Read the model definition and answer for the solid it produces. Units are mm, in the model's axes. Coordinates: 2 decimals unless noted, no trailing zeros. Write each loop counter-clockwise with the first axis right and the second up, starting at its lowest first coordinate (ties: lowest second). Pieces come first, ordered by that corner, then holes. Notation, with made-up numbers: (6, 14.5) -> (23, 14.5) arc R18 cw to (23, 41.5) -> close; hole circle Ø7 at (31.25, 54.25). An arc over 180 degrees is marked (long way). Answer in a Markdown table with one row per item. Add a question column.
Item 1: Section A-A on x = -75 is taken. Write down the section's boundary in (y, z), then the cut area to 3 significant figures.
Item 2: Given pin 1 Ø8 at (x, y) = (89.5, 55) entering from +Z; pin 2 Ø3 at (x, y) = (-90.5, 54) entering from +Z, each flat-ended and moving along its own axis, determine where each tip first touches the part or whether it passes through.
Item 3: Straight lines are drawn through the part: line 1 (Y direction, x = -90, z = 8.3); line 2 (Y direction, x = 25, z = 5.75); line 3 (X direction, y = 40.35, z = 3.5). For each, find the intervals that lie inside material, in ascending order. Write a range as from..to.
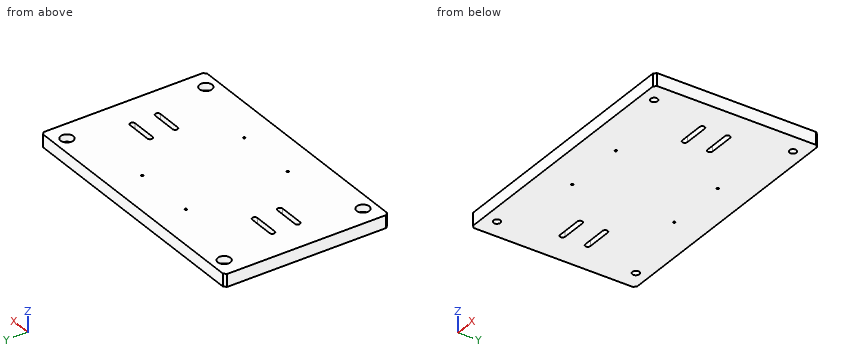
```python
from build123d import *

# Parameters (mm, degrees)
SKETCH1_W                                           = 210
SKETCH1_H                                           = 130
BOSS_EXTRUDE1_DEPTH                                 = 10
CUT_EXTRUDE1_DEPTH                                  = 124.895116934
CUT_EXTRUDE1_DEPTH_BACK                             = 124.895116934
HOLE_SIZE_PER_SOCKET_HEAD_CAP_SCREW_TYP_D           = 5.5
HOLE_SIZE_PER_SOCKET_HEAD_CAP_SCREW_TYP_CBORE_D     = 10
HOLE_SIZE_PER_SOCKET_HEAD_CAP_SCREW_TYP_CBORE_DEPTH = 5.7
M2_TAPPED_HOLE1_D                                   = 1.6
CHAMFER1_SIZE                                       = 2


with BuildPart() as part:
    # Sketch1 → Boss-Extrude1 (new body)
    with BuildSketch(Plane.XY):
        Rectangle(SKETCH1_W, SKETCH1_H)
    extrude(amount=BOSS_EXTRUDE1_DEPTH)

    # Sketch2 → Cut-Extrude1 (cut, two sides: drawn at the far end of the back side and taken through both)
    with BuildSketch(Plane.XY.offset(10).offset(-CUT_EXTRUDE1_DEPTH_BACK)):
        with BuildLine():
            Line((-80, 8), (-60, 8))
            ThreePointArc((-60, 8), (-58, 10), (-60, 12))
            Line((-60, 12), (-80, 12))
            ThreePointArc((-80, 12), (-82, 10), (-80, 8))
        make_face()
        with BuildLine():
            ThreePointArc((-60, -8), (-58, -10), (-60, -12))
            Line((-60, -12), (-80, -12))
            ThreePointArc((-80, -12), (-82, -10), (-80, -8))
            Line((-80, -8), (-60, -8))
        make_face()
        with BuildLine():
            Line((80, -8), (60, -8))
            ThreePointArc((60, -8), (58, -10), (60, -12))
            Line((60, -12), (80, -12))
            ThreePointArc((80, -12), (82, -10), (80, -8))
        make_face()
        with BuildLine():
            Line((80, 12), (60, 12))
            ThreePointArc((60, 12), (58, 10), (60, 8))
            Line((60, 8), (80, 8))
            ThreePointArc((80, 8), (82, 10), (80, 12))
        make_face()
    extrude(amount=CUT_EXTRUDE1_DEPTH + CUT_EXTRUDE1_DEPTH_BACK, mode=Mode.SUBTRACT)

    # Hole size (per socket head cap screw type)1 (through all)
    with Locations(Plane(origin=(-90, 55, 10), x_dir=(1, 0, 0), z_dir=(0, 0, 1))):
        with Locations((0, 0), (0, -110), (180, -110), (180, 0)):
            CounterBoreHole(HOLE_SIZE_PER_SOCKET_HEAD_CAP_SCREW_TYP_D / 2, HOLE_SIZE_PER_SOCKET_HEAD_CAP_SCREW_TYP_CBORE_D / 2, HOLE_SIZE_PER_SOCKET_HEAD_CAP_SCREW_TYP_CBORE_DEPTH)

    # M2 Tapped Hole1 (through all)
    with Locations(Plane(origin=(-25, 40.35, 10), x_dir=(1, 0, 0), z_dir=(0, 0, 1))):
        with Locations((0, 0), (50, 0), (50, -80.7), (0, -80.7)):
            Hole(M2_TAPPED_HOLE1_D / 2)

    # Chamfer1
    chamfer1_edges = [part.edges().sort_by_distance(p)[0] for p in [
        (105, -65, 5),
        (-105, -65, 5),
        (-105, 65, 5),
        (105, 65, 5),
    ]]
    chamfer(chamfer1_edges, length=CHAMFER1_SIZE)


solid = part.part
```
Results below:
| question | item | result |
|---|---|---|
| 1 | outline | (-65, 0) -> (-12, 0) -> (-12, 10) -> (-65, 10) -> close; (-8, 0) -> (8, 0) -> (8, 10) -> (-8, 10) -> close; (12, 0) -> (65, 0) -> (65, 10) -> (12, 10) -> close |
| 1 | area | 1,220 mm2 |
| 2 | pin 1 | stops at z = 4.3 |
| 2 | pin 2 | passes through |
| 3 | line 1 | y = -65..-60, -50..50, 60..65 |
| 3 | line 2 | y = -65..-41.15, -39.55..39.55, 41.15..65 |
| 3 | line 3 | x = -105..-25.8, -24.2..24.2, 25.8..105 |
